Source: CAD feature listing. Evaluate the final solid. Frame: model axes, mm. Face numbers are marked on the shaded views. A direction names the side the tool comes from. Round coordinates to 2 decimals unless told otherwise and drop trailing zeros. Order: outer loops, then holes, each group sorted by start corner. A loop starts at its lowest first (then second) coordinate and runs counter-clockwise, first axis right, second up. Notation, with made-up numbers: (75.5, 22.5) - (106.5, 22.5) arc R20 ccw to (106.5, 37.5) - close; hole circle Ø2 at (21.25, 32.5). An arc over 180 degrees is marked (long way). Put each result on its own line as item: value. Start each with the question number.
1) Access query for the marked faces 1 and 2. Directions: +Z, -Z, +X, -X, +Y, -Y. A direction counts if a zero-diameter tool reaches every point of the face in a straight line with its end or side. Return the directions, or none.
2) Mould query, pull axis X, two halves, no side actions, for the marked faces 3, 4 and 5. Classes: +X half, -X half, draft (parallel to the pull), parting line (faces both ways), or undercut.
3) Contact query for flat-ended pins moving along their axis: P1, Ø1.5, axis at y = -11, z = -15.5, coming from the -X side; P2, Ø11.5, axis at x = 0, z = 0, coming from the -Y side; P3, Ø1.5, axis at x = 3, y = -2.5, coming from the +Z side; P4, Ø1.5, axis at x = -10.5, y = -17.5, coming from the -Z side. Output: stop coordinate, or through.
4) Line query: probe 1 along Z at (x, y) = (3.5, -1.25); probe 2 along X at (y, z) = (-10, 7) (3 decimals); probe 3 along X at (y, z) = (-17.5, 3). Output: solid intervals per line, ascending. Write a range as [from, to].
5) Section C-C on y = -14. Output: boundary loops of the cut face in (x, z), then the cut area to 3 significant figures.
6) Section A-A on x = 0. Output: boundary loops of the cut face in (y, z).
7) Section B-B on y = -6.5. Output: boundary loops of the cut face in (x, z).
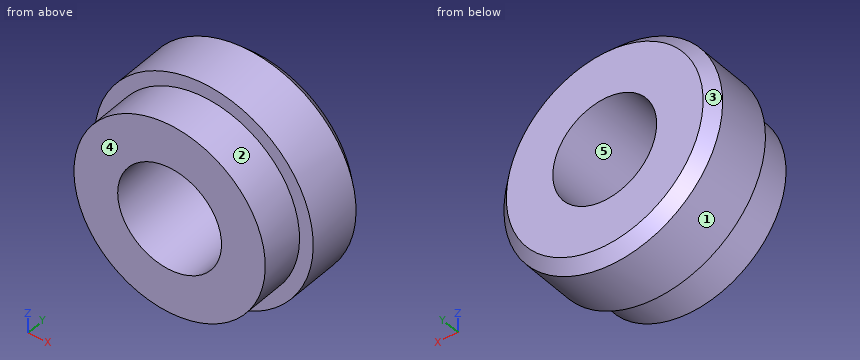
```python
from build123d import *

# Parameters (mm, degrees)
G1_2_TAPPED_HOLE1_D     = 19
G1_2_TAPPED_HOLE1_DEPTH = 47.35
G1_2_TAPPED_HOLE1_TIP   = 5.708175881
CHAMFER1_SIZE           = 2


with BuildPart() as part:
    # Sketch1 → Revolve1 (revolve)
    with BuildSketch(Plane.XY, mode=Mode.PRIVATE) as revolve1_sk:
        Polygon((0, 0), (20, 0), (20, -12), (17.5, -12), (17.5, -20), (0, -20), align=None)
    revolve(revolve1_sk.sketch.rotate(Axis((0, -20, 0), (0, 1, 0)), 90), axis=Axis((0, -20, 0), (0, 1, 0)))

    # G1/2 Tapped Hole1
    with Locations(Plane(origin=(0, 0, 0), x_dir=(1, 0, 0), z_dir=(0, 1, 0))):
        with Locations((0, 0)):
            Hole(G1_2_TAPPED_HOLE1_D / 2, depth=G1_2_TAPPED_HOLE1_DEPTH)
            with Locations((0, 0, -(G1_2_TAPPED_HOLE1_DEPTH + G1_2_TAPPED_HOLE1_TIP / 2))):  # 118° drill point
                Cone(0, G1_2_TAPPED_HOLE1_D / 2, G1_2_TAPPED_HOLE1_TIP, mode=Mode.SUBTRACT)

    # Chamfer1
    chamfer1_edges = [part.edges().sort_by_distance(p)[0] for p in [
        (0, 0, 20),
    ]]
    chamfer(chamfer1_edges, length=CHAMFER1_SIZE)


solid = part.part
```
Answer sheet:
1. face 1: +Y, -Y
1. face 2: -Y
2. face 3: parting line
2. face 4: draft
2. face 5: undercut
3. P1: x = -13.51
3. P2: through
3. P3: z = 19.87
3. P4: z = -14.53
4. probe 1: [-18.93, -8.83], [8.83, 18.93]
4. probe 2: [-18.735, -6.423], [6.423, 18.735]
4. probe 3: [-17.24, -9.01], [9.01, 17.24]
5. outline: circle Ø35 at (0, 0); hole circle Ø19 at (0, 0)
5. area: 679 mm^2
6. outline: (-20, -17.5) - (-12, -17.5) - (-12, -20) - (-2, -20) - (0, -18) - (0, -9.5) - (-20, -9.5) - close; (-20, 9.5) - (0, 9.5) - (0, 18) - (-2, 20) - (-12, 20) - (-12, 17.5) - (-20, 17.5) - close
7. outline: circle Ø40 at (0, 0); hole circle Ø19 at (0, 0)
